from build123d import *

# Parameters (mm, degrees)
HEAD_AND_SHANK_PROFILE_80_50_R   = 40
HEAD_AND_SHANK_PROFILE_80_50_R_2 = 25
HEAD_80_DEPTH                    = 30
SKETCH1_3_R                      = 25
SHANK_50_DEPTH                   = 120
HEAD_CHAMFER_10X45_SIZE          = 10
SHANK_END_CHAMFER_10X45_SIZE     = 10
CROSS_HOLE_PROFILE_R             = 6
CROSS_HOLE_12_DEPTH              = 30


with BuildPart() as part:
    # Head and Shank Profile _80-_50 → Head _80 (new body)
    # profile 1 of 2: a face of its own
    with BuildSketch(Plane.XY):
        Circle(HEAD_AND_SHANK_PROFILE_80_50_R)
        Circle(HEAD_AND_SHANK_PROFILE_80_50_R_2, mode=Mode.SUBTRACT)
    # profile 2 of 2: a face of its own
    with BuildSketch(Plane.XY):
        Circle(HEAD_AND_SHANK_PROFILE_80_50_R_2)
    extrude(amount=HEAD_80_DEPTH)

    # Sketch1_3 → Shank _50 (add)
    with BuildSketch(Plane.XY):
        with Locations(Location((0, 0, 0), (0, 0, 180))):
            Circle(SKETCH1_3_R)
    extrude(amount=SHANK_50_DEPTH)

    # Head Chamfer 10x45
    head_chamfer_10x45_edges = [part.edges().sort_by_distance(p)[0] for p in [
        (-40, 0, 0),
    ]]
    chamfer(head_chamfer_10x45_edges, length=HEAD_CHAMFER_10X45_SIZE)

    # Shank End Chamfer 10x45
    shank_end_chamfer_10x45_edges = [part.edges().sort_by_distance(p)[0] for p in [
        (25, 0, 120),
    ]]
    chamfer(shank_end_chamfer_10x45_edges, length=SHANK_END_CHAMFER_10X45_SIZE)

    # Cross Hole Profile → Cross Hole _12 (cut, symmetric)
    with BuildSketch(Plane(origin=(0, 0, 0), x_dir=(1, 0, 0), z_dir=(0, 1, 0))):
        with Locations(Location((0, -102, 0), (0, 0, 270))):
            Circle(CROSS_HOLE_PROFILE_R)
    extrude(amount=CROSS_HOLE_12_DEPTH, both=True, mode=Mode.SUBTRACT)


solid = part.part
Verification items for the finished model (mm, model axes). A direction names the side the tool comes from. Round coordinates to 2 decimals unless told otherwise and drop trailing zeros. Order: outer loops, then holes, each group sorted by start corner. A loop starts at its lowest first (then second) coordinate and runs counter-clockwise, first axis right, second up. Notation, with made-up numbers: (29, 42.25) -> (44, 42.25) arc R31 ccw to (44, 74.25) -> close; hole circle Ø7 at (-22.75, 20). An arc over 180 degrees is marked (long way). Put each result on its own line as item: value.
1) Section check A-A (x = 0). Record the cut outline in (y, z).
Final values:
outline: (-40, 10) -> (-30, 0) -> (30, 0) -> (40, 10) -> (40, 30) -> (25, 30) -> (25, 96) -> (-25, 96) -> (-25, 30) -> (-40, 30) -> close; (-25, 108) -> (25, 108) -> (25, 110) -> (15, 120) -> (-15, 120) -> (-25, 110) -> close
2) Set-up check for faces 1 (the conical face through (-3.987, 30.365, 0.626)), 2 (the cylindrical face through (-11.5, 22.2, 69.4)): record each of +Z, -Z, +X, -X, +Y, -Y from which the full face is reachable in a straight line by a thin tool's end or side.
Final values:
face 1: -Z
face 2: +Z
3) Section check B-B (y = 0). Record the cut outline in (x, z).
Final values:
outline: (-40, 10) -> (-30, 0) -> (30, 0) -> (40, 10) -> (40, 30) -> (25, 30) -> (25, 110) -> (15, 120) -> (-15, 120) -> (-25, 110) -> (-25, 30) -> (-40, 30) -> close; hole circle Ø12 at (0, 102)
4) Material ranges on line 1 (Z direction, x = 0, y = -9.5); line 2 (Z direction, x = 16.5, y = 19); line 3 (Z direction, x = -3, y = -14), recorded low to high.
Final values:
line 1: z = 0 to 96, 108 to 120
line 2: z = 0 to 30
line 3: z = 0 to 96.8, 107.2 to 120
5) Depth check by flat-ended pin: pin 1 (4 mm diameter, centred on y = -0.5, z = 59, fed in from -X); pin 2 (1 mm diameter, centred on x = 13.5, z = 60, fed in from +Y); pin 3 (2 mm diameter, centred on x = 2, z = 58.5, fed in from -Y); pin 4 (7 mm diameter, centred on x = 0, z = 102, fed in from -Y). Enter the tip coordinate at first touch or a pass-through.
Final values:
pin 1: stops at x = -25
pin 2: stops at y = 21.35
pin 3: stops at y = -24.98
pin 4: passes through
6) Section check C-C (z = 24). Record the cut outline in (x, y), then the cut area to 3 significant figures.
Final values:
outline: circle Ø80 at (0, 0)
area: 5,030 mm^2
7) Section check D-D (z = 97.5). Record the cut outline in (x, y), then the cut area to 3 significant figures.
Final values:
outline: (-3.97, -24.68) -> (-3.97, 24.68) arc R25 ccw to start; (3.97, -24.68) arc R25 ccw to (3.97, 24.68) -> close
area: 1,570 mm^2
